```python
from build123d import *

# Parameters (mm, degrees)
SKETCH1_R           = 2.5
BOSS_EXTRUDE1_DEPTH = 12
BOSS_EXTRUDE2_DEPTH = 2
CHAMFER1_SIZE       = 0.5


with BuildPart() as part:
    # Sketch1 → Boss-Extrude1 (new body)
    with BuildSketch(Plane.XY):
        with Locations((720, 45)):
            Circle(SKETCH1_R)
    extrude(amount=-BOSS_EXTRUDE1_DEPTH)

    # Sketch2 → Boss-Extrude2 (add)
    with BuildSketch(Plane.XY):
        Polygon((718.096078213, 41.702310731), (721.903921787, 41.702310731), (723.807843574, 45), (721.903921787, 48.297689269), (718.096078213, 48.297689269), (716.192156426, 45), align=None)
    extrude(amount=BOSS_EXTRUDE2_DEPTH)

    # Chamfer1
    chamfer1_edges = [part.edges().sort_by_distance(p)[0] for p in [
        (717.5, 45, -12),
        (717.144117319, 43.351155365, 2),
        (720, 41.702310731, 2),
        (722.855882681, 43.351155365, 2),
        (722.855882681, 46.648844635, 2),
        (720, 48.297689269, 2),
        (717.144117319, 46.648844635, 2),
    ]]
    chamfer(chamfer1_edges, length=CHAMFER1_SIZE)


solid = part.part
```
The listing builds one solid part. Answer for the finished solid, in the listing's coordinates (mm). A direction names the side the tool comes from. Give positions to 0.01 mm unless a question says otherwise; leave off trailing zeros. Loops run counter-clockwise (first coordinate to the right, second up) from the corner with the lowest first, then second, coordinate; pieces in that order, holes last. Notation, with made-up numbers: (-30, 43) - (-11, 43) arc R19 ccw to (-11, 78) - close; hole circle Ø8 at (16, -21). An arc over 180 degrees is marked (long way). Answer as CSV lines item,"result". Start each with the question number.
Item 1: For faces 1 (the face through (723, 45, 0)), 2 (the face through (722.869, 46.626, 0.74)), determine the directions among +Z, -Z, +X, -X, +Y, -Y from which every point of the face is accessible in a straight line to the end or side of a thin tool.
Item 2: Each of these flat-tipped pins is pushed along its axis until it touches: pin 1 (3 mm diameter, centred on y = 43.5, z = -6.5, fed in from -X); pin 2 (3 mm diameter, centred on x = 722, z = -9, fed in from +Y); pin 3 (1 mm diameter, centred on y = 44, z = -3.5, fed in from -X). Where does it stop, or does it pass through?
Item 3: A cutting plane is placed at B-B on z = -5.5. Determine the outline of the cut face in (x, y), then the cut area to 3 significant figures.
Item 4: Find the intervals of material crossed by line 1 (Z direction, x = 721.75, y = 42.5); line 2 (Y direction, x = 721.5, z = -6.25); line 3 (Y direction, x = 720.75, z = -4), in increasing order. Write a range as from..to.
Item 5: A cutting plane is placed at A-A on x = 720. Determine the outline of the cut face in (y, z), then the cut area to 3 significant figures.
Found:
1,face 1,"-Z"
1,face 2,"+Z, -Z, +X, +Y"
2,pin 1,"stops at x = 717.5"
2,pin 2,"stops at y = 47.45"
2,pin 3,"stops at x = 717.55"
3,outline,"circle Ø5 at (720, 45)"
3,area,"19.6 mm^2"
4,line 1,"z = 0..2"
4,line 2,"y = 43..47"
4,line 3,"y = 42.62..47.38"
5,outline,"(41.7, 0) - (42.5, 0) - (42.5, -11.5) - (43, -12) - (47, -12) - (47.5, -11.5) - (47.5, 0) - (48.3, 0) - (48.3, 1.5) - (47.8, 2) - (42.2, 2) - (41.7, 1.5) - close"
5,area,"72.7 mm^2"
